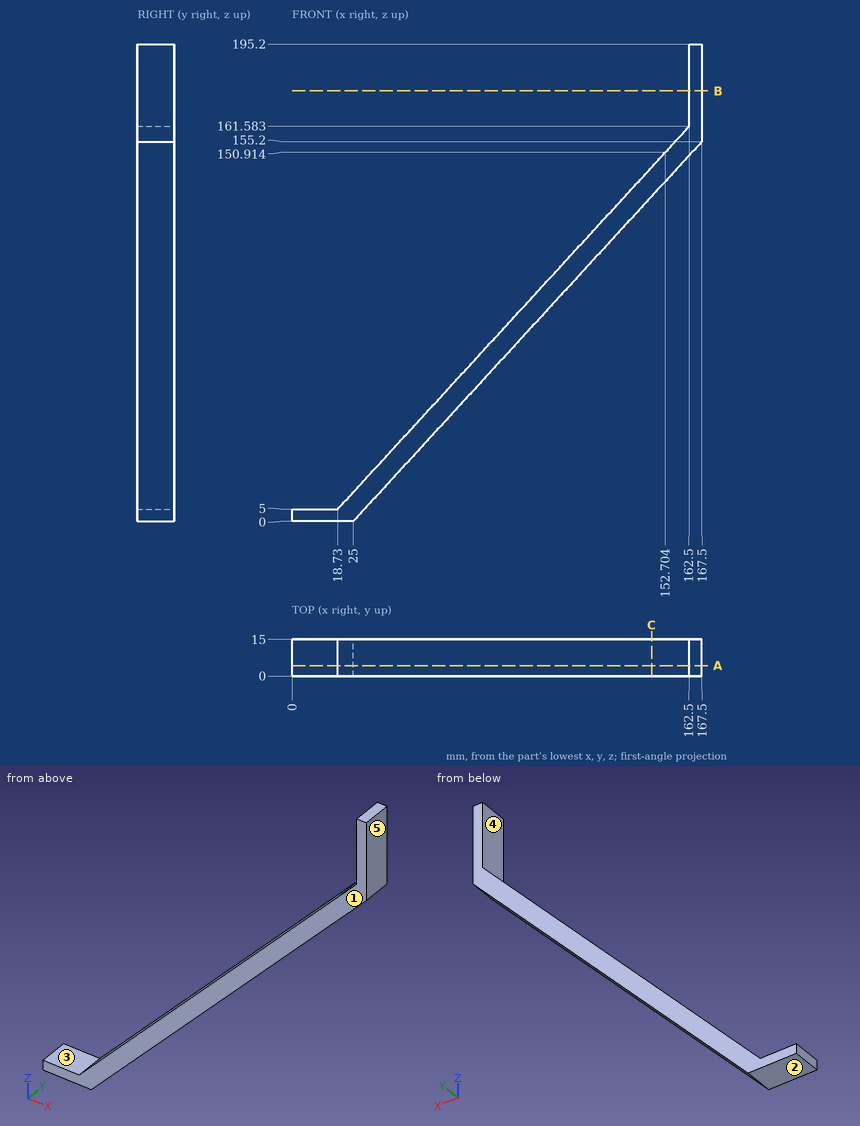
Print and shaded views of the part. All mm, measured from the part's lowest x, y and z. A direction names the side the tool comes from. Give positions to 0.01 mm unless a question says otherwise; leave off trailing zeros. Write each loop counter-clockwise with the first axis right and the second up, starting at its lowest first coordinate (ties: lowest second). Pieces come first, ordered by that corner, then holes. Notation, with made-up numbers: (50.5, 71) - (64.5, 71) arc R28 ccw to (64.5, 92) - close; hole circle Ø9 at (82, 43). An arc over 180 degrees is marked (long way). One line per question, with ' | ' between items. Start each with the question number.
(1) Wall check: line 1 along Z through (x, y) = (12, 11.75); line 2 along Z through (x, y) = (129, 5.75) (1 decimal); line 3 along X through (y, z) = (11.5, 94) (1 decimal). Give the ranges that are in metal, low to high. Write a range as from..to.
(2) Two-plate mould, pull along Z, no slides. Class the marked faces 1, 2 and 3: +Z half, -Z half, draft (parallel to the pull), parting line (faces both ways), or undercut.
(3) 3-axis set-ups, long thin cutter, end or side, ignore diameter. For the marked faces 4 and 5: which of +Z, -Z, +X, -X, +Y, -Y reach the whole face in a straight line?
(4) Pin check, flat tips, straight feed: P1, Ø6, axis at x = 30, y = 3.5, coming from the -Z side; P2, Ø1.5, axis at y = 6.5, z = 114, coming from the -X side; P3, Ø3, axis at x = 121, y = 1.5, coming from the -Z side. Stop position of each tip, or through.
(5) Slice it at A-A on y = 4.25. Write the cut outline in (x, z) (1 decimal), plus the area to 3 significant figures.
(6) Slice it at B-B on z = 176. Write the cut outline in (x, y), plus the area to 3 significant figures.
(7) Slice it at C-C on x = 147. Write the cut outline in (y, z).
Results below:
1) line 1: 0..5 | line 2: 113.3..125.1 | line 3: 100.4..111.3
2) face 1: draft | face 2: -Z half | face 3: +Z half
3) face 4: +Z, -X, +Y, -Y | face 5: +Z, -Z, +X, +Y, -Y
4) P1: z = 2.18 | P2: x = 118.12 | P3: z = 102.92
5) outline: (0, 0) - (25, 0) - (167.5, 155.2) - (167.5, 195.2) - (162.5, 195.2) - (162.5, 161.6) - (18.7, 5) - (0, 5) - close | area: 1,990 mm^2
6) outline: (162.5, 0) - (167.5, 0) - (167.5, 15) - (162.5, 15) - close | area: 75.0 mm^2
7) outline: (0, 132.87) - (15, 132.87) - (15, 144.7) - (0, 144.7) - close
